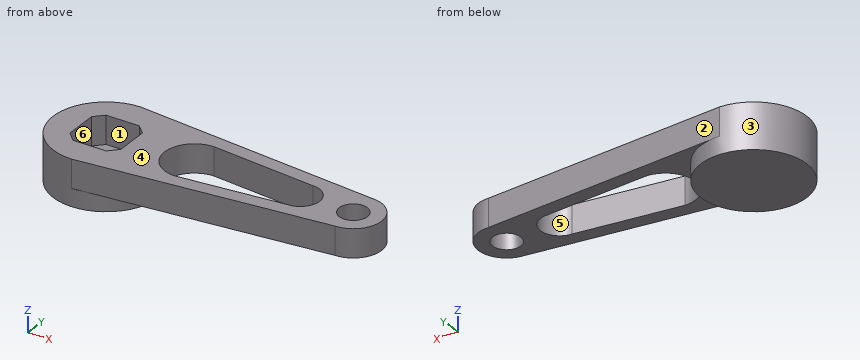
from build123d import *

# Parameters (mm, degrees)
LEVER_ARM_PLATE_DEPTH  = 8
TAPERED_SLOT_CUT_DEPTH = 8
HUB_START              = 5
HUB_BOSS_SKETCH_R      = 15
HUB_BOSS_DEPTH         = 5
PIN_HOLE_SKETCH_R      = 4
PIN_HOLE_DEPTH         = 8
HEX_SOCKET_CUT_DEPTH   = 8


with BuildPart() as part:
    # Lever Profile Sketch → Lever Arm Plate (new body)
    with BuildSketch(Plane.XY):
        with BuildLine():
            Line((0, 15), (70, 8))
            ThreePointArc((70, 8), (78, 0), (70, -8))
            Line((70, -8), (0, -15))
            ThreePointArc((0, -15), (-15, 0), (0, 15))
        make_face()
    extrude(amount=LEVER_ARM_PLATE_DEPTH)

    # Tapered Slot Sketch → Tapered Slot Cut (cut)
    with BuildSketch(Plane.XY.offset(8)):
        with BuildLine():
            Line((25, 8.44), (55, 5.45))
            ThreePointArc((55, 5.45), (60.45, 0), (55, -5.45))
            Line((55, -5.45), (25, -8.44))
            ThreePointArc((25, -8.44), (16.56, 0), (25, 8.44))
        make_face()
    extrude(amount=-TAPERED_SLOT_CUT_DEPTH, mode=Mode.SUBTRACT)

    # Hub Boss Sketch → Hub Boss (add)
    with BuildSketch(Plane(origin=(0, 0, 0), x_dir=(-1, 0, 0), z_dir=(0, 0, -1)).offset(HUB_START)):
        Circle(HUB_BOSS_SKETCH_R)
    extrude(amount=-HUB_BOSS_DEPTH)

    # Pin Hole Sketch → Pin Hole (cut)
    with BuildSketch(Plane.XY.offset(8)):
        with Locations((70, 0)):
            Circle(PIN_HOLE_SKETCH_R)
    extrude(amount=-PIN_HOLE_DEPTH, mode=Mode.SUBTRACT)

    # Hex Socket Sketch → Hex Socket Cut (cut)
    with BuildSketch(Plane.XY.offset(8)):
        Polygon((0, 7.21), (-4.71, 7.21), (-7.21, 4.71), (-7.21, -4.71), (-4.71, -7.21), (4.71, -7.21), (7.21, -4.71), (7.21, 4.71), (4.71, 7.21), align=None)
    extrude(amount=-HEX_SOCKET_CUT_DEPTH, mode=Mode.SUBTRACT)


solid = part.part
Input: part model. Units: mm. Frame: model coordinates. Face numbers are marked on the shaded views. A direction names the side the tool comes from. Coordinates: 2 decimals unless noted, no trailing zeros. Loops run counter-clockwise (first coordinate to the right, second up) from the corner with the lowest first, then second, coordinate; pieces in that order, holes last. Notation, with made-up numbers: (84, 7) -> (141, 7) arc R23 ccw to (141, 16) -> close; hole circle Ø2 at (64.25, -36.5). An arc over 180 degrees is marked (long way). Write item = value, one per line. Start each with the question number.
Item 1: Cut plane D-D, the plane z = -2.5. Return loops of the section in (x, y), plus the area to 3 significant figures.
Item 2: Material intervals for line 1 (Y direction, x = 70, z = 3.5); line 2 (Z direction, x = 15, y = 9); line 3 (Z direction, x = 4.5, y = 5.75), sorted ascending.
Item 3: First-contact query: P1, Ø14.5, axis at x = 40.5, y = 1.5, coming from the -Z side; P2, Ø4, axis at y = -2.5, z = 3.5, coming from the +X side; P3, Ø10.5, axis at x = 70, y = 0, coming from the +Z side; P4, Ø4.5, axis at x = 0.5, y = 2.5, coming from the +Z side. Flat tips, straight axial feed; report the tip coordinate or a pass-through.
Item 4: Reachability of the marked faces 4, 5 and 6 from +Z, -Z, +X, -X, +Y, -Y: full face, straight path, thin tool, end or side. Return the list, or none.
Item 5: Cut plane C-C, the plane x = 27.5. Return loops of the section in (y, z).
Item 6: Cut plane A-A, the plane z = 1.25. Return loops of the section in (x, y).
Item 7: Mould query, pull axis X, two halves, no side actions, for the marked faces 1, 2 and 3. Classes: pulls with the +X half, pulls with the -X half, needs draft (parallel to the pull), parting line crosses it, or undercut.
Ans:
q1.outline = circle Ø30 at (0, 0)
q1.area = 707 mm²
q2.line_1 = -8 to -4, 4 to 8
q2.line_2 = 0 to 8
q2.line_3 = -5 to 0
q3.P1 = 0
q3.P2 = 77.98
q3.P3 = 8
q3.P4 = 0
q4.face_4 = +Z, +X, -X, +Y, -Y
q4.face_5 = +Z, -Z
q4.face_6 = +Z
q5.outline = (-12.25, 0) -> (-8.19, 0) -> (-8.19, 8) -> (-12.25, 8) -> close; (8.19, 0) -> (12.25, 0) -> (12.25, 8) -> (8.19, 8) -> close
q6.outline = (0, -15) -> (70, -8) arc R8 ccw to (70, 8) -> (0, 15) arc R15 ccw to start; hole (-7.21, -4.71) -> (-4.71, -7.21) -> (4.71, -7.21) -> (7.21, -4.71) -> (7.21, 4.71) -> (4.71, 7.21) -> (-4.71, 7.21) -> (-7.21, 4.71) -> close; hole (25, -8.44) -> (55, -5.45) arc R5.45 ccw to (55, 5.45) -> (25, 8.44) arc R8.44 ccw to start; hole circle Ø8 at (70, 0)
q7.face_1 = undercut
q7.face_2 = pulls with the +X half
q7.face_3 = parting line crosses it
